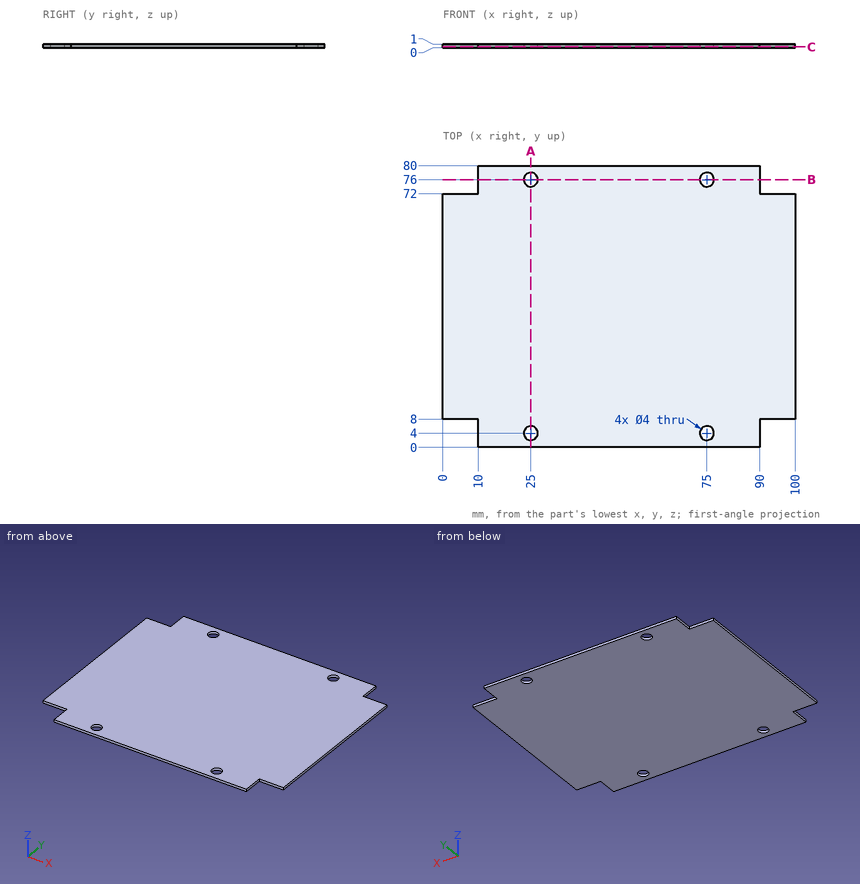
Geometry: see drawing. Coordinates: mm, zero at the bounding-box minimum. Coordinates: 2 decimals unless noted, no trailing zeros. Order: outer loops, then holes, each group sorted by start corner. A loop starts at its lowest first (then second) coordinate and runs counter-clockwise, first axis right, second up. Notation, with made-up numbers: M 75.5,74 L 123.5,74 A28 cw 123.5,105 Z; hole C 56.5,44.5 d5. An arc over 180 degrees is marked long. Answer in a Markdown table with one row per item. Add a question column.
Q1. Section query A-A on x = 25. Return the cut outline in (y, z).
Q2. Section query C-C on z = 0.2. Return the cut outline in (x, y).
Q3. Line query: L1, parallel to X at y = 76, z = 0.75; L2, parallel to Y at x = 25, z = 0.7; L3, parallel to Y at x = 76, z = 0.7. Output: solid intervals per line, ascending.
Q4. Section query B-B on y = 76. Return the cut outline in (x, z), and give its area (3 significant figures).
Q5. Contact query for a flat-ended pin moving along its axis: P1, Ø0.5, axis at x = 3.5, z = 0.5, coming from the -Y side. Output: stop coordinate, or through.
Completed:
| question | item | result |
|---|---|---|
| 1 | outline | M 0,0 L 2,0 L 2,1 L 0,1 Z; M 6,0 L 74,0 L 74,1 L 6,1 Z; M 78,0 L 80,0 L 80,1 L 78,1 Z |
| 2 | outline | M 0,8 L 10,8 L 10,0 L 90,0 L 90,8 L 100,8 L 100,72 L 90,72 L 90,80 L 10,80 L 10,72 L 0,72 Z; hole C 25,4 d4; hole C 25,76 d4; hole C 75,4 d4; hole C 75,76 d4 |
| 3 | L1 | x = 10 to 23, 27 to 73, 77 to 90 |
| 3 | L2 | y = 0 to 2, 6 to 74, 78 to 80 |
| 3 | L3 | y = 0 to 2.27, 5.73 to 74.27, 77.73 to 80 |
| 4 | outline | M 10,0 L 23,0 L 23,1 L 10,1 Z; M 27,0 L 73,0 L 73,1 L 27,1 Z; M 77,0 L 90,0 L 90,1 L 77,1 Z |
| 4 | area | 72.0 mm2 |
| 5 | P1 | stops at y = 8 |
